CAD build for the part. Positions are in the model's coordinates, mm. A direction names the side the tool comes from. Coordinates: 2 decimals unless noted, no trailing zeros. Loops run counter-clockwise (first coordinate to the right, second up) from the corner with the lowest first, then second, coordinate; pieces in that order, holes last.
1) Pin check, flat tips, straight feed: pin 1 Ø24 at (x, z) = (16, 0) entering from +Y; pin 2 Ø1 at (x, z) = (16, -7) entering from -Y; pin 3 Ø24 at (x, y) = (-1.5, 6.5) entering from -Z. Stop position of each tip, or through.
2) Which spindle directions (+Z, -Z, +X, -X, +Y, -Y) get a long thin tool onto all of the face, cutting with end or side? Do faces 5 (the flat face through (0, -10, 0)), 6 (the flat face through (-0.5, 10.2, 15)), 7 (the flat face through (61, 0, 28)). Say none if no direction does.
3) Saw through at A-A, the plane z = -18. Write the cut outline in (x, y), and give its area (3 significant figures).
4) Saw through at D-D, the plane z = -10. Write the cut outline in (x, y), and give its area (3 significant figures).
5) Wall check: line 1 along X through (y, z) = (-36, -24); line 2 along X through (y, z) = (6, -13); line 3 along Y through (x, z) = (19.5, -6.5). Give the ranges that are in metal, low to high.
6) Saw through at B-B, the plane x = 7.5. Write the cut outline in (y, z), and give its area (3 significant figures).
7) Saw through at C-C, the plane y = 34. Write the cut outline in (x, z), and give its area (3 significant figures).
8) Two-plate mould, pull along Y, no slides. Class faces 1 (the flat face through (40, -1, 0)), 2 (the flat face through (0, -15, 0)), 3 (the flat face through (-0.5, 10.2, -15)), 4 (the flat face through (60, 1, 0)): +Y half, -Y half, draft (parallel to the pull), parting line (faces both ways), or undercut.
```python
from build123d import *

# Parameters (mm, degrees)
CENTER_WEB_DEPTH     = 15
WEB_WINDOW_CUT_DEPTH = 80
SIDE_LOOP_DEPTH      = 28


with BuildPart() as part:
    # Center Web Profile → Center Web (new, symmetric)
    with BuildSketch(Plane.XY):
        Polygon((35, 0), (35, 15), (-35, 15), (-35, -15), (35, -15), align=None)
    extrude(amount=CENTER_WEB_DEPTH, both=True)

    # Web Window Profile 40x20 → Web Window Cut (cut)
    with BuildSketch(Plane.XY.offset(15)):
        with BuildLine():
            Line((-20, 10), (20, 10))
            ThreePointArc((20, 10), (30, 0), (20, -10))
            Line((20, -10), (-20, -10))
            ThreePointArc((-20, -10), (-30, 0), (-20, 10))
        make_face()
    extrude(amount=-WEB_WINDOW_CUT_DEPTH, mode=Mode.SUBTRACT)

    # Side Loop Profile → Side Loop (add, symmetric)
    with BuildSketch(Plane.XY):
        with BuildLine():
            Line((35, 0), (35, 45))
            ThreePointArc((35, 45), (50, 60), (65, 45))
            Line((65, 45), (65, -45))
            ThreePointArc((65, -45), (50, -60), (35, -45))
            Line((35, -45), (35, -15))
            Line((35, -15), (35, 0))
        make_face()
        with BuildLine():
            Line((60, 45), (60, -45))
            ThreePointArc((60, -45), (50, -55), (40, -45))
            Line((40, -45), (40, 45))
            ThreePointArc((40, 45), (50, 55), (60, 45))
        make_face(mode=Mode.SUBTRACT)
    side_loop = extrude(amount=SIDE_LOOP_DEPTH, both=True)

    # Side Loop Mirror: Side Loop across plane
    add(side_loop.mirror(Plane(origin=(0, 0, 0), x_dir=(0, 0, 1), z_dir=(1, 0, 0))))


solid = part.part
```
Data:
1. pin 1: stops at y = 15
1. pin 2: stops at y = -15
1. pin 3: stops at z = -15
2. face 5: +Z, -Z
2. face 6: +Z, +Y, -Y
2. face 7: +Z, +X, -X, +Y, -Y
3. outline: (-65, -45) arc R15 ccw to (-35, -45) - (-35, 45) arc R15 ccw to (-65, 45) - close; (35, -45) arc R15 ccw to (65, -45) - (65, 45) arc R15 ccw to (35, 45) - close; hole (-60, -45) arc R10 ccw to (-40, -45) - (-40, 45) arc R10 ccw to (-60, 45) - close; hole (40, -45) arc R10 ccw to (60, -45) - (60, 45) arc R10 ccw to (40, 45) - close
3. area: 2,590 mm2
4. outline: (-65, -45) arc R15 ccw to (-35, -45) - (-35, -15) - (35, -15) - (35, -45) arc R15 ccw to (65, -45) - (65, 45) arc R15 ccw to (35, 45) - (35, 15) - (-35, 15) - (-35, 45) arc R15 ccw to (-65, 45) - close; hole (-60, -45) arc R10 ccw to (-40, -45) - (-40, 45) arc R10 ccw to (-60, 45) - close; hole (-20, -10) - (20, -10) arc R10 ccw to (20, 10) - (-20, 10) arc R10 ccw to start; hole (40, -45) arc R10 ccw to (60, -45) - (60, 45) arc R10 ccw to (40, 45) - close
4. area: 3,570 mm2
5. line 1: x = -65 to -60, -40 to -35, 35 to 40, 60 to 65
5. line 2: x = -65 to -60, -40 to -28, 28 to 40, 60 to 65
5. line 3: y = -15 to -10, 10 to 15
6. outline: (-15, -15) - (-10, -15) - (-10, 15) - (-15, 15) - close; (10, -15) - (15, -15) - (15, 15) - (10, 15) - close
6. area: 300 mm2
7. outline: (-65, -28) - (-60, -28) - (-60, 28) - (-65, 28) - close; (-40, -28) - (-35, -28) - (-35, 28) - (-40, 28) - close; (35, -28) - (40, -28) - (40, 28) - (35, 28) - close; (60, -28) - (65, -28) - (65, 28) - (60, 28) - close
7. area: 1,120 mm2
8. face 1: undercut
8. face 2: -Y half
8. face 3: draft
8. face 4: undercut
